The drawing under review shows one solid part. Ordinate dimensions are in mm from its lowest x, y, z. A direction names the side the tool comes from. Coordinates: 2 decimals unless noted, no trailing zeros. Order: outer loops, then holes, each group sorted by start corner. A loop starts at its lowest first (then second) coordinate and runs counter-clockwise, first axis right, second up. Notation, with made-up numbers: (65, 30) -> (95, 30) arc R30 ccw to (95, 57) -> close; hole circle Ø3 at (79.5, 18). An arc over 180 degrees is marked (long way). Use a Markdown table: item, result. Add a question column.
Q1. Wall thickness on probe 1 along X at (y, z) = (36, 2.25); probe 2 along Y at (x, z) = (40.5, 1.5); probe 3 along Y at (x, z) = (37, 3.75): over which ranges is each line inside the solid? List them lowest first.
Q2. Add section C-C (x = 37). State the section outline as (y, z) points.
Q3. Machinability: for the marked faces 1 and 2, which of the approach directions +Z, -Z, +X, -X, +Y, -Y give a long, thin tool a straight path to every point of the face, cutting with its end or side? Answer none if there is none.
Q4. The part is to be moulded in two halves that separate along X. For the marked faces 3, 4 and 5, say which applies: pulls with the +X half, pulls with the -X half, needs draft (parallel to the pull), parting line crosses it, or undercut.
Q5. Add section A-A (y = 14.5). State the section outline as (x, z) points, then the cut area to 3 significant figures.
Q6. Add section B-B (z = 3). State the section outline as (x, y) points, then the cut area to 3 significant figures.
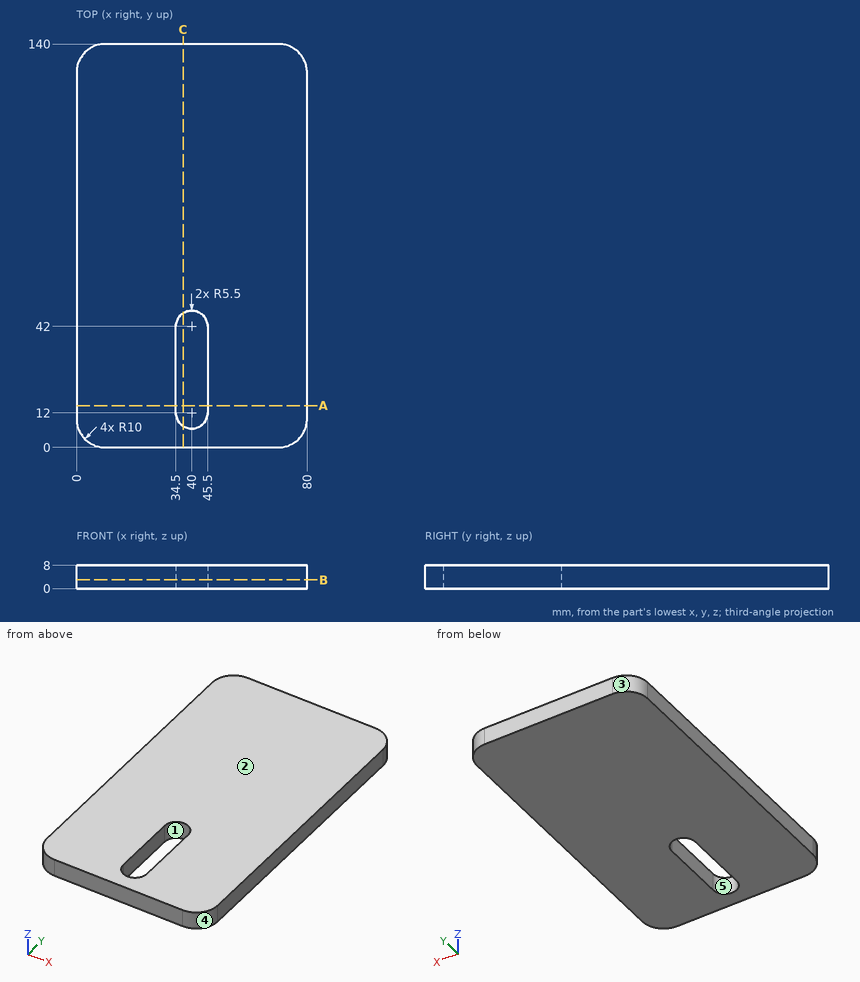
Established:
| question | item | result |
|---|---|---|
| 1 | probe 1 | 0 to 34.5, 45.5 to 80 |
| 1 | probe 2 | 0 to 6.52, 47.48 to 140 |
| 1 | probe 3 | 0 to 7.39, 46.61 to 140 |
| 2 | outline | (0, 0) -> (7.39, 0) -> (7.39, 8) -> (0, 8) -> close; (46.61, 0) -> (140, 0) -> (140, 8) -> (46.61, 8) -> close |
| 3 | face 1 | +Z, -Z |
| 3 | face 2 | +Z, +X, -X, +Y, -Y |
| 4 | face 3 | pulls with the -X half |
| 4 | face 4 | pulls with the +X half |
| 4 | face 5 | undercut |
| 5 | outline | (0, 0) -> (34.5, 0) -> (34.5, 8) -> (0, 8) -> close; (45.5, 0) -> (80, 0) -> (80, 8) -> (45.5, 8) -> close |
| 5 | area | 552 mm^2 |
| 6 | outline | (0, 10) arc R10 ccw to (10, 0) -> (70, 0) arc R10 ccw to (80, 10) -> (80, 130) arc R10 ccw to (70, 140) -> (10, 140) arc R10 ccw to (0, 130) -> close; hole (34.5, 12) arc R5.5 ccw to (45.5, 12) -> (45.5, 42) arc R5.5 ccw to (34.5, 42) -> close |
| 6 | area | 10,700 mm^2 |
